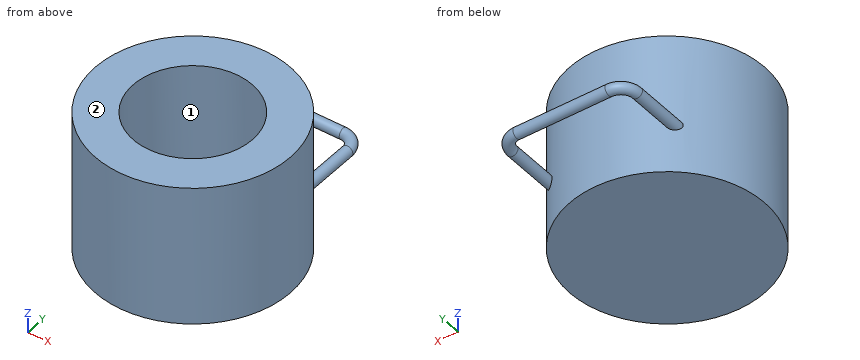
```python
from build123d import *

# Parameters (mm, degrees)
SKETCH1_R           = 90
BOSS_EXTRUDE1_DEPTH = 130
SKETCH2_R           = 55
CUT_EXTRUDE1_DEPTH  = 100
SWEEP1_PROFILE_R    = 5


with BuildPart() as part:
    # Sketch1 → Boss-Extrude1 (new body)
    with BuildSketch(Plane.XY):
        Circle(SKETCH1_R)
    extrude(amount=BOSS_EXTRUDE1_DEPTH)

    # Sketch2 → Cut-Extrude1 (cut)
    with BuildSketch(Plane.XY.offset(130)):
        Circle(SKETCH2_R)
    extrude(amount=-CUT_EXTRUDE1_DEPTH, mode=Mode.SUBTRACT)

    # Sweep1: sweep along a path in Sketch3
    with BuildLine(Plane(origin=(0, 0, 45), x_dir=(-1, 0, 0), z_dir=(0, 0, -1))) as sweep1_path:
        Line((-57.6, 56.789164475), (-57.6, 115.589164475))
        ThreePointArc((-57.6, 115.589164475), (-53.206601718, 126.195766193), (-42.6, 130.589164475))
        Line((-42.6, 130.589164475), (42.6, 130.589164475))
        ThreePointArc((42.6, 130.589164475), (53.206601718, 126.195766193), (57.6, 115.589164475))
        Line((57.6, 115.589164475), (57.6, 56.789164475))
    # Sweep1 profile (on start of the path) → Sweep1 (sweep)
    with BuildSketch(Plane(origin=(57.6, 56.789164475, 45), x_dir=(0, 0, 1), z_dir=(0, 1, 0))):
        Circle(SWEEP1_PROFILE_R)
    sweep(path=sweep1_path.line)


solid = part.part
```
Input: part model. Units: mm. Frame: model coordinates. Face numbers are marked on the shaded views. Give positions to 0.01 mm unless a question says otherwise; leave off trailing zeros. Loops run counter-clockwise (first coordinate to the right, second up) from the corner with the lowest first, then second, coordinate; pieces in that order, holes last. Notation, with made-up numbers: M 7,49.5 L 27,49.5 A16 cw 27,67.5 Z; hole C 18.25,14 d9. An arc over 180 degrees is marked long. Answer as CSV lines item,"result". Start each with the question number.
1. Section B-B on y = 0. Return loops of the section in (x, z), plus the area to 3 significant figures.
2. Section C-C on z = 67. Return loops of the section in (x, y), plus the area to 3 significant figures.
3. Pull-direction query (Y, two-part tool) for the marked faces 1 and 2; classes: released by +Y, released by -Y, zero draft, split by the parting line, or undercut.
4. Line query: L1, parallel to Y at x = 0, z = 79; L2, parallel to Z at x = 2.5, y = 18; L3, parallel to Y at x = -42, z = 117. Output: solid intervals per line, ascending.
5. Section A-A on x = 0. Return loops of the section in (y, z), plus the area to 3 significant figures.
6. Pin query (flat end, axial travel): P1, Ø10, axis at y = 9.5, z = 46.5, coming from the +X side; P2, Ø5, axis at x = 18, y = -44, coming from the +Z side; P3, Ø1.5, axis at x = -47.5, z = 85.5, coming from the -Y side. Return the tip coordinate at first contact, or that it passes through.
7. Section D-D on z = 45. Return loops of the section in (x, y).
Computed values:
1,outline,"M -90,0 L 90,0 L 90,130 L 55,130 L 55,30 L -55,30 L -55,130 L -90,130 Z"
1,area,"12,400 mm²"
2,outline,"C 0,0 d180; hole C 0,0 d110"
2,area,"15,900 mm²"
3,face 1,"undercut"
3,face 2,"zero draft"
4,L1,"y = -90 to -55, 55 to 90"
4,L2,"z = 0 to 30"
4,L3,"y = -79.6 to -35.51, 35.51 to 79.6"
5,outline,"M -90,0 L 90,0 L 90,130 L 55,130 L 55,30 L -55,30 L -55,130 L -90,130 Z; C 130.59,45 d10"
5,area,"12,500 mm²"
6,P1,"stops at x = 89.89"
6,P2,"stops at z = 30"
6,P3,"stops at y = -76.91"
7,outline,"M -62.6,64.66 A90 ccw long 62.6,64.66 L 62.6,115.59 A20 ccw 42.6,135.59 L -42.6,135.59 A20 ccw -62.6,115.59 Z; hole C 0,0 d110; hole M -52.6,73.03 A90 cw 52.6,73.03 L 52.6,115.59 A10 ccw 42.6,125.59 L -42.6,125.59 A10 ccw -52.6,115.59 Z"
